```python
from build123d import *

# Parameters (mm, degrees)
SKETCH_1_W                   = 18
SKETCH_1_H                   = 30
EXTRUDE_1_DEPTH              = 1700
CHAMFER_1_SIZE               = 2
HOLE_WIZARD_M8_1_D           = 9
HOLE_WIZARD_M8_1_CBORE_D     = 15
HOLE_WIZARD_M8_1_CBORE_DEPTH = 19


with BuildPart() as part:
    # 草图1 → 凸台-拉伸1 (new body)
    with BuildSketch(Plane(origin=(0, 0, 0), x_dir=(1, 0, 0), z_dir=(0, 1, 0))):
        with Locations((9, 15)):
            Rectangle(SKETCH_1_W, SKETCH_1_H)
    extrude(amount=EXTRUDE_1_DEPTH)

    # 倒角1
    chamfer_1_edges = [part.edges().sort_by_distance(p)[0] for p in [
        (18, 1700, -15),
        (0, 1700, -15),
        (18, 0, -15),
        (0, 0, -15),
    ]]
    chamfer(chamfer_1_edges, length=CHAMFER_1_SIZE)

    # M8 六角圆柱头螺钉的柱形沉头孔1 (through all)
    with Locations(Plane(origin=(0, 0, -30), x_dir=(-1, 0, 0), z_dir=(0, 0, -1))):
        with Locations((-9, 1600), (-9, 1350), (-9, 1100), (-9, 600), (-9, 350), (-9, 100), (-9, 850)):
            CounterBoreHole(HOLE_WIZARD_M8_1_D / 2, HOLE_WIZARD_M8_1_CBORE_D / 2, HOLE_WIZARD_M8_1_CBORE_DEPTH)


solid = part.part
```
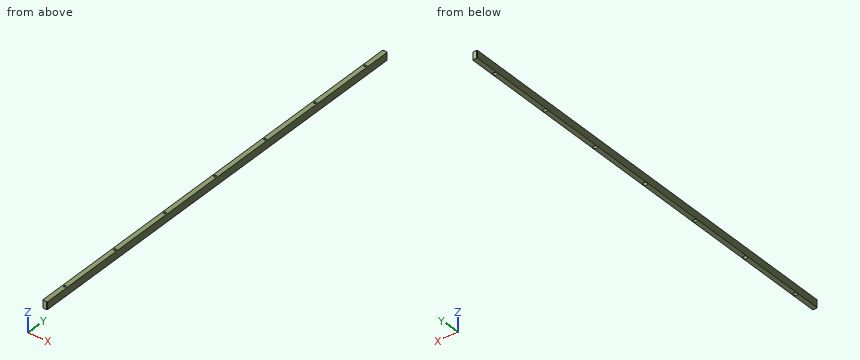
Can you work these out from the model? Positions are in its coordinate system, mm. Coordinates: 2 decimals unless noted, no trailing zeros. Loops run counter-clockwise (first coordinate to the right, second up) from the corner with the lowest first, then second, coordinate; pieces in that order, holes last. Notation, with made-up numbers: M 37,64.25 L 63,64.25 A34 cw 63,97.25 Z; hole C 24.5,69 d4. An arc over 180 degrees is marked long. Put each result on its own line as item: value. Start each with the question number.
(1) Imagine slicing it at B-B on x = 9. Give the number of separate pieces and of enclosed holes in the cut face, and give its area (3 significant figures).
(2) Will these pins go through, and if not, where does the flat tip stop? pin 1 Ø4.5 at (x, y) = (9.5, 1099) entering from -Z; pin 2 Ø4.5 at (x, y) = (12.5, 1348) entering from -Z.
(3) I need wall thicknesses on probe 1 along X at (y, z) = (1600, -2.5); probe 2 along X at (y, z) = (1350, -16.5); probe 3 along Z at (x, y) = (13.75, 1602). Which ranges of each line are inside material? Lowest first, please.
(4) Imagine slicing it at A-A on z = -24.5. List the corners of the cut face in (x, y) for me, and give its area (3 significant figures).
Worked answers:
1. separate pieces: 8
1. enclosed holes: 0
1. area: 48,300 mm2
2. pin 1: passes through
2. pin 2: stops at z = -11
3. probe 1: x = 0 to 4.5, 13.5 to 18
3. probe 2: x = 0 to 1.5, 16.5 to 18
3. probe 3: z = -11 to 0
4. outline: M 0,2 L 2,0 L 16,0 L 18,2 L 18,1698 L 16,1700 L 2,1700 L 0,1698 Z; hole C 9,100 d15; hole C 9,350 d15; hole C 9,600 d15; hole C 9,850 d15; hole C 9,1100 d15; hole C 9,1350 d15; hole C 9,1600 d15
4. area: 29,400 mm2
